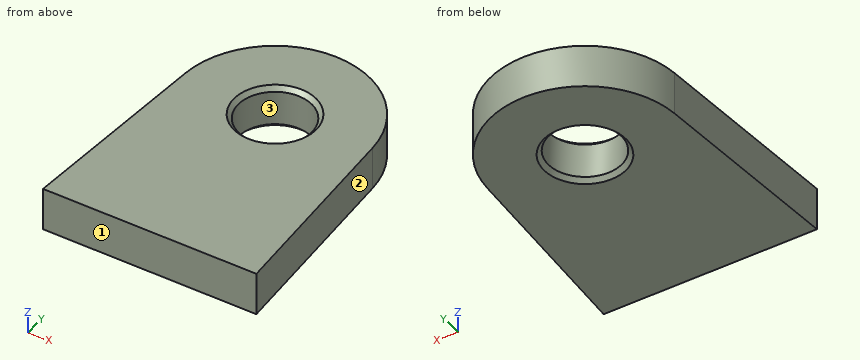
```python
from build123d import *

# Parameters (mm, degrees)
SKETCH1_R           = 8.5
BOSS_EXTRUDE1_DEPTH = 10
CHAMFER1_SIZE       = 1


with BuildPart() as part:
    # Sketch1 → Boss-Extrude1 (new body)
    with BuildSketch(Plane.XY):
        with BuildLine():
            Line((0, 0), (50, 0))
            Line((50, 0), (46.952793231, 46.440440684))
            ThreePointArc((46.952793231, 46.440440684), (25, 67), (3.047206769, 46.440440684))
            Line((3.047206769, 46.440440684), (0, 0))
        make_face()
        with Locations((25, 45)):
            Circle(SKETCH1_R, mode=Mode.SUBTRACT)
    extrude(amount=BOSS_EXTRUDE1_DEPTH)

    # Chamfer1
    chamfer1_edges = [part.edges().sort_by_distance(p)[0] for p in [
        (16.5, 45, 0),
        (16.5, 45, 10),
    ]]
    chamfer(chamfer1_edges, length=CHAMFER1_SIZE)


solid = part.part
```
CAD build for the part. Positions are in the model's coordinates, mm. Face numbers are marked on the shaded views. Round coordinates to 2 decimals unless told otherwise and drop trailing zeros. Write each loop counter-clockwise with the first axis right and the second up, starting at its lowest first coordinate (ties: lowest second). Pieces come first, ordered by that corner, then holes. Notation, with made-up numbers: M 87.5,3.5 L 131.5,3.5 A11 ccw 131.5,13.5 Z; hole C 88.25,-39.5 d4. An arc over 180 degrees is marked long. One line per question, with ' | ' between items.
1. Probe L1, parallel to Y at x = 25, z = 3.5; L2, parallel to Y at x = 31.5, z = 2; L3, parallel to X at y = 47, z = 6.75. List the from-to ranges inside material, lowest first. Write a range as from..to.
Working result:
L1: 0..36.5, 53.5..67 | L2: 0..39.52, 50.48..66.02 | L3: 3.09..16.74, 33.26..46.91
2. Cut at B-B on z = 8. Write the cut outline in (x, y).
Working result:
outline: M 0,0 L 50,0 L 46.95,46.44 A22 ccw 3.05,46.44 Z; hole C 25,45 d17
3. Pin check, flat tips, straight feed: pin 1 Ø3 at (y, z) = (52, 4) entering from +X; pin 2 Ø1 at (y, z) = (43.5, 6) entering from +X; pin 3 Ø4 at (x, z) = (37.5, 6.5) entering from +Y. Stop position of each tip, or through.
Working result:
pin 1: x = 46.3 | pin 2: x = 47.18 | pin 3: y = 64.33
4. Cut at A-A on x = 25. Write the cut outline in (y, z), and give its area (3 significant figures).
Working result:
outline: M 0,0 L 35.5,0 L 36.5,1 L 36.5,9 L 35.5,10 L 0,10 Z; M 53.5,1 L 54.5,0 L 67,0 L 67,10 L 54.5,10 L 53.5,9 Z | area: 498 mm2
5. Cut at D-D on y = 19.5. Write the cut outline in (x, z).
Working result:
outline: M 1.28,0 L 48.72,0 L 48.72,10 L 1.28,10 Z
6. Mould opens along X. For the marked faces 1, 2 and 3 say: pulls with the +X half, pulls with the -X half, needs draft (parallel to the pull), parting line crosses it, or undercut.
Working result:
face 1: needs draft | face 2: pulls with the +X half | face 3: undercut
7. Cut at C-C on y = 45. Write the cut outline in (x, z), and give its area (3 significant figures).
Working result:
outline: M 2.95,0 L 15.5,0 L 16.5,1 L 16.5,9 L 15.5,10 L 2.95,10 Z; M 33.5,1 L 34.5,0 L 47.05,0 L 47.05,10 L 34.5,10 L 33.5,9 Z | area: 269 mm2
